from build123d import *

# Parameters (mm, degrees)
SKETCH1_R                                        = 15
SKETCH1_W                                        = 100
SKETCH1_H                                        = 220
BOSS_EXTRUDE1_DEPTH                              = 30
CBORE_FOR_M8_PAN_HEAD_MACHINE_SCREW3_D           = 9
CBORE_FOR_M8_PAN_HEAD_MACHINE_SCREW3_CBORE_D     = 18
CBORE_FOR_M8_PAN_HEAD_MACHINE_SCREW3_CBORE_DEPTH = 6
SKETCH_1_R                                       = 5
CUT_EXTRUDE1_DEPTH                               = 20
SKETCH2_R                                        = 2
CUT_EXTRUDE2_DEPTH                               = 289.097205818


with BuildPart() as part:
    # Sketch1 → Boss-Extrude1 (new body)
    with BuildSketch(Plane(origin=(0, 0, 0), x_dir=(1, 0, 0), z_dir=(0, 1, 0))):
        with BuildLine():
            Line((-110, -250), (80, -250))
            Line((80, -250), (80, 30))
            Line((80, 30), (-110, 30))
            ThreePointArc((-110, 30), (-140, 0), (-110, -30))
            Line((-110, -30), (-110, -190))
            ThreePointArc((-110, -190), (-140, -220), (-110, -250))
        make_face()
        with Locations(Location((-110, 0, 0), (0, 0, 270))):
            Circle(SKETCH1_R, mode=Mode.SUBTRACT)
        with Locations(Location((-110, -220, 0), (0, 0, 270))):
            Circle(SKETCH1_R, mode=Mode.SUBTRACT)
        with Locations((0, -110)):
            Rectangle(SKETCH1_W, SKETCH1_H, mode=Mode.SUBTRACT)
    boss_extrude1 = extrude(amount=BOSS_EXTRUDE1_DEPTH)

    # CBORE for M8 Pan Head Machine Screw3 (through all)
    with Locations(Plane(origin=(0, 0, 0), x_dir=(-1, 0, 0), z_dir=(0, -1, 0))):
        with Locations((60, -230), (-60, -230), (-60, 10), (60, 10)):
            CounterBoreHole(CBORE_FOR_M8_PAN_HEAD_MACHINE_SCREW3_D / 2, CBORE_FOR_M8_PAN_HEAD_MACHINE_SCREW3_CBORE_D / 2, CBORE_FOR_M8_PAN_HEAD_MACHINE_SCREW3_CBORE_DEPTH)

    # Mirror1: Boss-Extrude1 across plane
    add(boss_extrude1.mirror(Plane(origin=(0, 0, 0), x_dir=(0, 0, 1), z_dir=(1, 0, 0))))

    # 草图1 → Cut-Extrude1 (cut)
    with BuildSketch(Plane(origin=(0, 30, 0), x_dir=(1, 0, 0), z_dir=(0, 1, 0))):
        with Locations(Location((-60, 13.06497659, 0), (0, 0, 270))):
            Circle(SKETCH_1_R)
        with Locations(Location((-60, -226.93502341, 0), (0, 0, 270))):
            Circle(SKETCH_1_R)
        with Locations(Location((60, 13.06497659, 0), (0, 0, 90))):
            Circle(SKETCH_1_R)
        with Locations(Location((60, -226.93502341, 0), (0, 0, 90))):
            Circle(SKETCH_1_R)
    extrude(amount=-CUT_EXTRUDE1_DEPTH, mode=Mode.SUBTRACT)

    # Sketch2 → Cut-Extrude2 (cut, through all)
    with BuildSketch(Plane(origin=(0, 30, 0), x_dir=(1, 0, 0), z_dir=(0, 1, 0))):
        with Locations(Location((-60, -21.93502341, 0), (0, 0, 270))):
            Circle(SKETCH2_R)
        with Locations(Location((60, -191.93502341, 0), (0, 0, 270))):
            Circle(SKETCH2_R)
    extrude(amount=-CUT_EXTRUDE2_DEPTH, mode=Mode.SUBTRACT)


solid = part.part
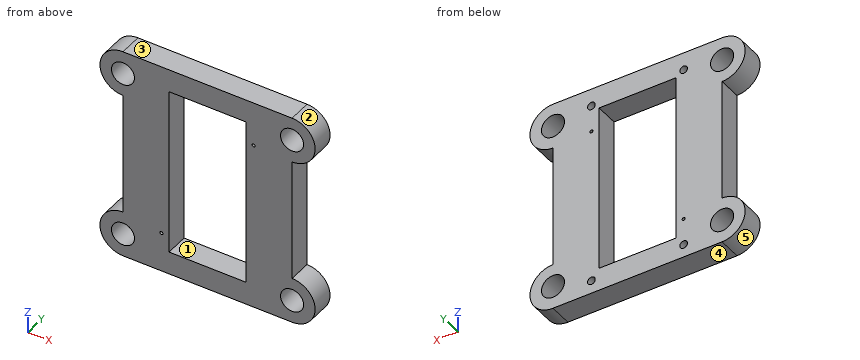
Could you check a few things on this model? Use its own coordinates, in mm. Face numbers are marked on the shaded views. A direction names the side the tool comes from. Give positions to 0.01 mm unless a question says otherwise; leave off trailing zeros. Loops run counter-clockwise (first coordinate to the right, second up) from the corner with the lowest first, then second, coordinate; pieces in that order, holes last. Notation, with made-up numbers: (-36.5, 53) -> (22.5, 53) arc R31 ccw to (22.5, 79) -> close; hole circle Ø11 at (56.25, -35). An arc over 180 degrees is marked (long way). Return JSON: item names as keys, results as strings.
Item 1: I need wall thicknesses on L1, parallel to Z at x = 108.5, y = 5.75; L2, parallel to X at y = 22.5, z = 220.5; L3, parallel to X at y = 7.25, z = 128.5. Which ranges of each line are inside material? Lowest first, please. Write a range as from..to.
Geometry results:
{"L1": "z = -30..-14.92, 14.92..205.08, 234.92..250", "L2": "x = -140..-124.99, -95.01..95.01, 124.99..140", "L3": "x = -110..-50, 50..110"}
Item 2: If we section it at B-B on y = 25.25: Count the separate pieces of the cut face and the enclosed holes in it, plus the area to 3 significant figures.
Geometry results:
{"separate pieces": "1", "enclosed holes": "11", "area": "42,100 mm²"}
Item 3: We'd pull the mould along Z, two halves only. Please class the marked faces 3, 4 and 5: +Z half, -Z half, draft (parallel to the pull), parting line (faces both ways), or undercut.
Geometry results:
{"face 3": "+Z half", "face 4": "-Z half", "face 5": "undercut"}
Item 4: I'm going to push flat-ended pins straight in: pin 1 (12 mm diameter, centred on y = 21.5, z = 181.5, fed in from +X); pin 2 (3 mm diameter, centred on x = -60, z = 21.94, fed in from -Y); pin 3 (3 mm diameter, centred on x = -60.5, z = -11, fed in from +Y); pin 4 (5 mm diameter, centred on y = 17, z = 213.5, fed in from +X). Where does each tip first touch, or does it pass through?
Geometry results:
{"pin 1": "stops at x = 110", "pin 2": "passes through", "pin 3": "stops at y = 10", "pin 4": "stops at x = 139.73"}
Item 5: If we section it at A-A on x = 25: List the corners of the cut face in (y, z) for me, plus the area to 3 significant figures.
Geometry results:
{"outline": "(0, -30) -> (30, -30) -> (30, 0) -> (0, 0) -> close; (0, 220) -> (30, 220) -> (30, 250) -> (0, 250) -> close", "area": "1,800 mm²"}
Item 6: Which directions (+Z, -Z, +X, -X, +Y, -Y) give clear straight access to the entire face, cutting with the end or side of a thin tool? Please do the marked faces 1 and 2.
Geometry results:
{"face 1": "+Y, -Y", "face 2": "+X, +Y, -Y"}
